The model under review builds one solid part; all positions refer to its coordinate system, in mm. A direction names the side the tool comes from. Give positions to 0.01 mm unless a question says otherwise; leave off trailing zeros. Write each loop counter-clockwise with the first axis right and the second up, starting at its lowest first coordinate (ties: lowest second). Pieces come first, ordered by that corner, then holes. Notation, with made-up numbers: M 56.5,56 L 92.5,56 A30 ccw 92.5,87 Z; hole C 3,22 d11. An arc over 180 degrees is marked long. Write each question's results on one line, items separated by ' | '. Start each with the question number.
from build123d import *
from build123d.topology import SkipClean

# Parameters (mm, degrees)
SKETCH1_R               = 10
SKETCH1_R_2             = 7.5
BOSS_EXTRUDE1_DEPTH     = 45
CUT_EXTRUDE1_DEPTH      = 48.16990566
CUT_EXTRUDE1_DEPTH_BACK = 48.16990566
SKETCH2_R               = 3
SKETCH3_R               = 12.5
BOSS_EXTRUDE2_DEPTH     = 20
CUT_EXTRUDE2_DEPTH      = 49.347699108
CUT_EXTRUDE2_DEPTH_BACK = 49.347699108


with BuildPart() as part:
    # Sketch1 → Boss-Extrude1 (new body)
    with BuildSketch(Plane.XY):
        with Locations(Location((0, 0, 0), (0, 0, 180))):
            Circle(SKETCH1_R)
        with Locations(Location((0, 0, 0), (0, 0, 180))):
            Circle(SKETCH1_R_2, mode=Mode.SUBTRACT)
    extrude(amount=BOSS_EXTRUDE1_DEPTH)

    # Sketch2 → Cut-Extrude1 (cut, two sides: drawn at the far end of the back side and taken through both)
    with BuildSketch(Plane(origin=(0, 0, 0), x_dir=(1, 0, 0), z_dir=(0, 1, 0)).offset(-CUT_EXTRUDE1_DEPTH_BACK)):
        with Locations(Location((0, -30, 0), (0, 0, 270))):
            Circle(SKETCH2_R)
    extrude(amount=CUT_EXTRUDE1_DEPTH + CUT_EXTRUDE1_DEPTH_BACK, mode=Mode.SUBTRACT)

    # Sketch3 → Boss-Extrude2 (add)
    with BuildSketch(Plane(origin=(0, 0, 0), x_dir=(-1, 0, 0), z_dir=(0, 0, -1))):
        Circle(SKETCH3_R)
    extrude(amount=BOSS_EXTRUDE2_DEPTH)

    # Sketch4 → Cut-Extrude2 (cut, two sides: drawn at the far end of the back side and taken through both)
    with BuildSketch(Plane(origin=(0, 0, 0), x_dir=(1, 0, 0), z_dir=(0, 1, 0)).offset(-CUT_EXTRUDE2_DEPTH_BACK)):
        Polygon((0, 20), (12.5, 20), (12.5, 0), (10, -10), (0, 0), align=None)
    extrude(amount=CUT_EXTRUDE2_DEPTH + CUT_EXTRUDE2_DEPTH_BACK, mode=Mode.SUBTRACT)

    # Sketch5 → Cut-Revolve3 (revolve, cut)
    with SkipClean():  # the faces are left unmerged after this step: merging them gives an invalid solid
        with BuildSketch(Plane(origin=(0, 0, 0), x_dir=(1, 0, 0), z_dir=(0, 1, 0))):
            with BuildLine():
                Line((0, 17.5), (0, 2.5))
                ThreePointArc((0, 2.5), (-7.5, 10), (0, 17.5))
            make_face()
        revolve(axis=Axis((0, 0, 0), (0, 0, -1)), mode=Mode.SUBTRACT)


solid = part.part
(1) Add section D-D (x = 5.25). State the section outline as (y, z) points, then the cut area to 3 significant figures.
(2) Machinability: for faces 5 (the flat face through (-10, 2, 0)), 6 (the flat face through (-4, -7, 45)), 7 (the flat face through (0, 8, -10)), 8 (the cylindrical face through (-9.237, 3.83, 22.185)), which of the approach directions +Z, -Z, +X, -X, +Y, -Y give a long, thin tool a straight path to every point of the face, cutting with its end or side? Answer none if there is none.
(3) Add section B-B (z = 30). State the section outline as (x, y) points.
(4) Add section A-A (y = 1.25). State the section outline as (x, z) points.
(5) Clearance check with flat-ended pins moving along their axes: P1, Ø2, axis at x = 0.5, z = 3, coming from the +Y side; P2, Ø2, axis at y = -9, z = -1.5, coming from the +X side; P3, Ø3, axis at x = 7.5, y = -8, coming from the -Z side; P4, Ø3.5, axis at x = 0, z = 30, coming from the +Y side. State where each tip first meets the part, or that it passes through.
(6) Draft analysis for pull direction Z (two halves, no side actions). For faces 1 (the flat face through (-3, 0, 0)), 2 (the flat face through (7.3, -2.4, 7.3)), 3 (the cylindrical face through (-1.15, -8.46, 32.77)), 4 (the cylindrical face through (-12.497, -0.275, -9.86)), state which applies: pulls with the +Z half, pulls with the -Z half, needs draft (parallel to the pull), parting line crosses it, or undercut.
(7) Add section C-C (x = -1.5). State the section outline as (y, z) points, then the cut area to 3 significant figures.
(8) Wall thickness on L1, parallel to Y at x = 0, z = 8.5; L2, parallel to X at y = 8.5, z = 30; L3, parallel to Z at x = -10.5, y = 6: over which ranges is each line inside the solid? List them lowest first.
Calculated:
1) outline: M -8.51,5.25 L -5.36,5.25 L -5.36,45 L -8.51,45 Z; M 5.36,5.25 L 8.51,5.25 L 8.51,45 L 5.36,45 Z | area: 251 mm²
2) face 5: +Z, -X | face 6: +Z, +X, -X, +Y, -Y | face 7: -Z, +X, +Y, -Y | face 8: +Z
3) outline: M -3,-9.54 L -3,-6.87 A7.5 cw -3,6.87 L -3,9.54 A10 ccw Z; M 3,-9.54 A10 ccw 3,9.54 L 3,6.87 A7.5 cw 3,-6.87 Z
4) outline: M -12.44,-20 L 0,-20 L 0,-17.4 A7.4 cw 0,-2.6 L 0,0 L -7.4,0 L -7.4,45 L -9.92,45 L -9.92,0 L -12.44,0 Z; M 7.4,7.4 L 9.92,9.92 L 9.92,45 L 7.4,45 Z
5) P1: stops at y = 10 | P2: stops at x = 0 | P3: stops at z = 6 | P4: passes through
6) face 1: pulls with the +Z half | face 2: pulls with the -Z half | face 3: undercut | face 4: needs draft
7) outline: M -12.41,-20 L 12.41,-20 L 12.41,0 L 9.89,0 L 9.89,27.4 L 7.35,27.4 L 7.35,0 L -7.35,0 L -7.35,27.4 L -9.89,27.4 L -9.89,0 L -12.41,0 Z; M -9.89,32.6 L -7.35,32.6 L -7.35,45 L -9.89,45 Z; M 7.35,32.6 L 9.89,32.6 L 9.89,45 L 7.35,45 Z; hole C 0,-10 d14.7 | area: 529 mm²
8) L1: y = -10 to -7.5, 7.5 to 10 | L2: x = -5.27 to -3, 3 to 5.27 | L3: z = -20 to 0
